```python
from build123d import *

# Parameters (mm, degrees)
BOSS_EXTRUDE1_DEPTH = 12
SKETCH2_R           = 4
BOSS_EXTRUDE2_DEPTH = 20
SKETCH3_W           = 32
SKETCH3_H           = 10
CUT_EXTRUDE1_DEPTH  = 20
SKETCH4_R           = 3
CUT_EXTRUDE2_DEPTH  = 34
CHAMFER1_SIZE       = 1


with BuildPart() as part:
    # Sketch1 → Boss-Extrude1 (new, symmetric)
    with BuildSketch(Plane(origin=(0, 0, 0), x_dir=(1, 0, 0), z_dir=(0, 1, 0))):
        with BuildLine():
            Line((-8, 0), (-8, -11))
            Line((-8, -11), (8, -11))
            Line((8, -11), (8, 0))
            ThreePointArc((8, 0), (0, 8), (-8, 0))
        make_face()
    extrude(amount=BOSS_EXTRUDE1_DEPTH, both=True)

    # Sketch2 → Boss-Extrude2 (add)
    with BuildSketch(Plane.XY.offset(11)):
        with Locations(Location((0, 0, 0), (0, 0, 180))):
            Circle(SKETCH2_R)
    extrude(amount=BOSS_EXTRUDE2_DEPTH)

    # Sketch3 → Cut-Extrude1 (cut)
    with BuildSketch(Plane(origin=(8, 0, 0), x_dir=(0, 0, -1), z_dir=(1, 0, 0))):
        with Locations((8, 0)):
            Rectangle(SKETCH3_W, SKETCH3_H)
    extrude(amount=-CUT_EXTRUDE1_DEPTH, mode=Mode.SUBTRACT)

    # Sketch4 → Cut-Extrude2 (cut)
    with BuildSketch(Plane.XZ.offset(12)):
        with Locations(Location((0, 0, 0), (0, 0, 270))):
            Circle(SKETCH4_R)
    extrude(amount=-CUT_EXTRUDE2_DEPTH, mode=Mode.SUBTRACT)

    # Chamfer1
    chamfer1_edges = [part.edges().sort_by_distance(p)[0] for p in [
        (4, 0, 31),
    ]]
    chamfer(chamfer1_edges, length=CHAMFER1_SIZE)


solid = part.part
```
CAD build for the part. Positions are in the model's coordinates, mm. A direction names the side the tool comes from. Round coordinates to 2 decimals unless told otherwise and drop trailing zeros. Write each loop counter-clockwise with the first axis right and the second up, starting at its lowest first coordinate (ties: lowest second). Pieces come first, ordered by that corner, then holes.
Item 1: Band-saw the part on B-B on y = 0. Write the cut outline in (x, z).
Filled in:
outline: (-8, 8) - (8, 8) - (8, 11) - (4, 11) - (4, 30) - (3, 31) - (-3, 31) - (-4, 30) - (-4, 11) - (-8, 11) - close
Item 2: Tool access for faces 1 (the flat face through (0, 5, 4)), 2 (the flat face through (-0.1, 12, 3.5)), 3 (the cylindrical face through (0.867, 3.905, 20.367)): list every direction of +Z, -Z, +X, -X, +Y, -Y with a clear straight run to the whole face (end or side of a thin tool).
Filled in:
face 1: -Z, +X, -X
face 2: +Z, -Z, +X, -X, +Y
face 3: +Z
Item 3: Mould opens along Z. For faces 4 (the flat face through (0, 0, 8)), 5 (the cylindrical face through (0.9, 8.45, -2.86)), 6 (the flat face through (0, -5, 4)) say: released by +Z, released by -Z, zero draft, split by the parting line, or undercut.
Filled in:
face 4: released by -Z
face 5: undercut
face 6: zero draft
Item 4: Band-saw the part on C-C on x = 0. Write the cut outline in (y, z).
Filled in:
outline: (-12, -8) - (-5, -8) - (-5, -3) - (-12, -3) - close; (-12, 3) - (-5, 3) - (-5, 8) - (5, 8) - (5, 3) - (12, 3) - (12, 11) - (4, 11) - (4, 30) - (3, 31) - (-3, 31) - (-4, 30) - (-4, 11) - (-12, 11) - close; (5, -8) - (12, -8) - (12, -3) - (5, -3) - close
Item 5: Band-saw the part on A-A on z = 6.5. Write the cut outline in (x, y), then the cut area to 3 significant figures.
Filled in:
outline: (-8, -12) - (8, -12) - (8, -5) - (-8, -5) - close; (-8, 5) - (8, 5) - (8, 12) - (-8, 12) - close
area: 224 mm2
Item 6: Band-saw the part on D-D on y = -8.5. Write the cut outline in (x, z).
Filled in:
outline: (-8, 0) arc R8 ccw to (8, 0) - (8, 11) - (-8, 11) - close; hole circle Ø6 at (0, 0)
Item 7: Drop flat-ended pins along their axis: pin 1 Ø8 at (x, y) = (4.5, -4.5) entering from -Z; pin 2 Ø3 at (x, y) = (-4, 1) entering from -Z; pin 3 Ø8 at (y, z) = (6.5, 16.5) entering from +X. Give the stop position or say it passes through.
Filled in:
pin 1: stops at z = -7.98
pin 2: stops at z = 8
pin 3: stops at x = 3.12
Item 8: Drill centre lines: L1, parallel to Y at x = -1.75, z = -2.5; L2, parallel to X at y = -7, z = 0; L3, parallel to Z at x = 4.5, y = 1.5. Where is each one in solid material? Low to high.
Filled in:
L1: y = -12 to -5, 5 to 12
L2: x = -8 to -3, 3 to 8
L3: z = 8 to 11
